Verification items for this drawing (mm, ordinates from the low corner). A direction names the side the tool comes from. Coordinates: 2 decimals unless noted, no trailing zeros. Write each loop counter-clockwise with the first axis right and the second up, starting at its lowest first coordinate (ties: lowest second). Pieces come first, ordered by that corner, then holes. Notation, with made-up numbers: M -15,-0.75 L 43,-0.75 A5 ccw 43,4.25 Z; hole C -9.5,-19 d10. An arc over 180 degrees is marked long. Put each result on its own line as item: value. Start each with the question number.
1) Cross-section at C-C on y = 10. Record the cut outline in (x, z), plus the area to 3 significant figures.
2) Gauge pin test, flat ends, axial feed: pin 1 (12 mm diameter, centred on y = 17, z = 5.5, fed in from -X); pin 2 (4 mm diameter, centred on x = 16.5, z = 20, fed in from -Y); pin 3 (6 mm diameter, centred on x = 19, y = 24, fed in from +Z). Record the tip position at first contact, or that the pin passes through.
3) Cross-section at B-B on z = 12. Record the cut outline in (x, y), plus the area to 3 significant figures.
4) Set-up check for the marked faces 1, 2 and 3: record each of +Z, -Z, +X, -X, +Y, -Y from which the full face is reachable in a straight line by a thin tool's end or side.
5) Cross-section at A-A on x = 12. Record the cut outline in (y, z).
6) Scan lines: line 1 along Y through (x, z) = (3.5, 14); line 2 along Z through (x, y) = (11.5, 19); line 3 along Z through (x, y) = (12, 73.5). Record each from-to range of solid material in increasing order.
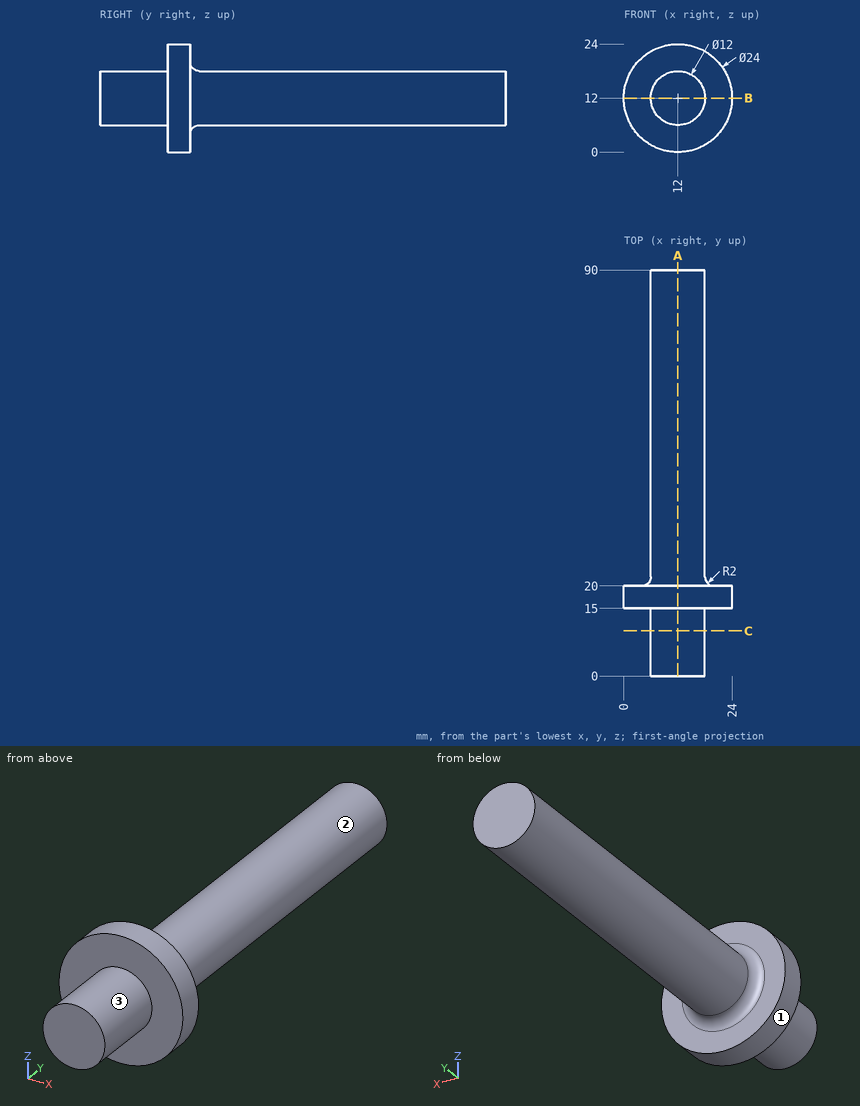
Answer key:
1. outline: C 12,12 d12
1. area: 113 mm²
2. pin 1: stops at x = 0.01
2. pin 2: stops at y = 15
2. pin 3: stops at z = 16.47
3. outline: M 0,15 L 6,15 L 6,0 L 18,0 L 18,15 L 24,15 L 24,20 L 20,20 A2 cw 18,22 L 18,90 L 6,90 L 6,22 A2 cw 4,20 L 0,20 Z
3. area: 1,140 mm²
4. face 1: +Y, -Y
4. face 2: +Y
4. face 3: -Y
5. outline: M 0,6 L 15,6 L 15,0 L 20,0 L 20,4 A2 cw 22,6 L 90,6 L 90,18 L 22,18 A2 cw 20,20 L 20,24 L 15,24 L 15,18 L 0,18 Z
6. line 1: y = 15 to 20
6. line 2: z = 0.01 to 23.99
6. line 3: z = 6 to 18
